```python
from build123d import *
from build123d.topology import SkipClean

# Parameters (mm, degrees)
EXTRUDE_1_DEPTH          = 12.5
HOLE_WIZARD_M14_1_D      = 12
HOLE_WIZARD_M14_1_DEPTH  = 18
SKETCH_7_W               = 66
SKETCH_7_H               = 25
EXTRUDE_2_DEPTH          = 12
CUT_EXTRUDE_1_DEPTH      = 156.608483059
CUT_EXTRUDE_1_DEPTH_BACK = 156.608483059
SKETCH_14_W              = 30
SKETCH_14_H              = 25
EXTRUDE_START            = -12.5
EXTRUDE_3_DEPTH          = 7.5
SKETCH_8_4_R             = 38.5
SKETCH_8_4_R_2           = 36.5
EXTRUDE_1_2_DEPTH        = 7.5
FILLET_1_R               = 1


with BuildPart() as part:
    # 草图1 → Extrude 1 (new, symmetric)
    with BuildSketch(Plane.XY):
        Polygon((-33, -150), (-15, -150), (-15, -100), (0, -100), (15, -100), (15, -150), (33, -150), (33, 90), (15, 90), (-15, 90), (-33, 90), align=None)
    extrude(amount=EXTRUDE_1_DEPTH, both=True)

    # M14 螺纹孔1
    with Locations(Plane(origin=(33, -131.5, 0.451602972), x_dir=(0, 0, 1), z_dir=(1, 0, 0))):
        with Locations((0, 0)):
            hole_wizard_m14_1 = Hole(HOLE_WIZARD_M14_1_D / 2, depth=HOLE_WIZARD_M14_1_DEPTH)

    # 镜向1: M14 螺纹孔1 across plane
    add(hole_wizard_m14_1.mirror(Plane(origin=(0, 0, 0), x_dir=(0, 0, 1), z_dir=(1, 0, 0))), mode=Mode.SUBTRACT)

    # 草图7 → 凸台-拉伸2 (add)
    with BuildSketch(Plane(origin=(0, 90, 0), x_dir=(1, 0, 0), z_dir=(0, 1, 0))):
        Rectangle(SKETCH_7_W, SKETCH_7_H)
    extrude(amount=EXTRUDE_2_DEPTH)

    # 草图14 → 切除-拉伸1 (cut, two sides: drawn at the far end of the back side and taken through both)
    with BuildSketch(Plane(origin=(0, 0, -12.5), x_dir=(-1, 0, 0), z_dir=(0, 0, -1)).offset(-CUT_EXTRUDE_1_DEPTH_BACK)):
        with Locations((0, 84.064537633)):
            Rectangle(SKETCH_14_W, SKETCH_14_H)
    extrude(amount=CUT_EXTRUDE_1_DEPTH + CUT_EXTRUDE_1_DEPTH_BACK, mode=Mode.SUBTRACT)

    # 草图8 → 凸台-拉伸3 (add, symmetric)
    with BuildSketch(Plane(origin=(0, 0, -12.5), x_dir=(-1, 0, 0), z_dir=(0, 0, -1)).offset(EXTRUDE_START)):
        with BuildLine():
            Line((-33, 102), (0, 102))
            Line((0, 102), (0, 125))
            ThreePointArc((0, 125), (-25.809397513, 135.690602487), (-36.5, 161.5))
            Line((-36.5, 161.5), (-36.5, 102))
            Line((-36.5, 102), (-33, 102))
        make_face()
        with BuildLine():
            Line((0, 102), (33, 102))
            Line((33, 102), (36.5, 102))
            Line((36.5, 102), (36.5, 161.5))
            ThreePointArc((36.5, 161.5), (25.809397513, 135.690602487), (0, 125))
            Line((0, 125), (0, 102))
        make_face()
    extrude(amount=EXTRUDE_3_DEPTH, both=True)

    # 草图8<4> → Extrude 1 2 (add, symmetric)
    with SkipClean():  # the faces are left unmerged after this step: merging them gives an invalid solid
        with BuildSketch(Plane(origin=(0, 0, -12.5), x_dir=(-1, 0, 0), z_dir=(0, 0, -1)).offset(EXTRUDE_START)):
            with Locations((0, 161.5)):
                Circle(SKETCH_8_4_R)
            with Locations((0, 161.5)):
                Circle(SKETCH_8_4_R_2, mode=Mode.SUBTRACT)
        extrude(amount=EXTRUDE_1_2_DEPTH, both=True)

    # 圆角1
    fillet_1_edges = [part.edges().sort_by_distance(p)[0] for p in [
        (0, 102, -7.5),
        (0, 102, 7.5),
    ]]
    fillet(fillet_1_edges, radius=FILLET_1_R)


solid = part.part
```
Could you check a few things on this model? Use its own coordinates, in mm. A direction names the side the tool comes from. Give positions to 0.01 mm unless a question says otherwise; leave off trailing zeros. Loops run counter-clockwise (first coordinate to the right, second up) from the corner with the lowest first, then second, coordinate; pieces in that order, holes last. Notation, with made-up numbers: (-21, 60) - (-16, 60) arc R23 ccw to (-16, 74) - close; hole circle Ø3 at (30.25, -15.75). An arc over 180 degrees is marked (long way). Use one line per item in the form item = value.
1. Thinking about a two-plate mould opening in X: for faces 4 (the face through (-15, -125, 0)), 5 (the face through (24, -150, 0)), 6 (the face through (-36.5, 125, 0)), which applies, released by +X, released by -X, zero draft, split by the parting line, or undercut?
Response values:
face_4 = undercut
face_5 = zero draft
face_6 = released by -X
2. On a 3-axis mill with a long thin cutter (end or side, diameter ignored), from which of +Z, -Z, +X, -X, +Y, -Y can I reach the whole of each face in a straight line? I mean faces 1 (the face through (0, -100, 0)), 2 (the face through (23.874, -125.643, 1.752)), 3 (the face through (15, 84, 0)). Say none if no direction works.
Response values:
face_1 = +Z, -Z, -Y
face_2 = +X, -X
face_3 = +Z, -Z
3. I need wall thicknesses on probe 1 along X at (y, z) = (-118, -2); probe 2 along Z at (x, y) = (-29.5, -131.5); probe 3 along Y at (x, z) = (-6.5, -9). Which ranges of each line are inside material? Lowest first, please.
Response values:
probe_1 = -33 to -15, 15 to 33
probe_2 = -12.5 to -5.55, 6.45 to 12.5
probe_3 = -100 to 71.56, 96.56 to 102
4. I want a section at C-C (x = 20). Please give me the cut outline in (y, z), and give its area (3 significant figures).
Response values:
outline = (-150, -12.5) - (102, -12.5) - (102, -8.5) arc R1 cw to (103, -7.5) - (130.97, -7.5) - (130.97, 7.5) - (103, 7.5) arc R1 cw to (102, 8.5) - (102, 12.5) - (-150, 12.5) - close; (192.03, -7.5) - (194.4, -7.5) - (194.4, 7.5) - (192.03, 7.5) - close; hole circle Ø12 at (-131.5, 0.45)
area = 6,660 mm²
5. I want a section at A-A (y = -131.5). Please give me the cut outline in (x, z), and give its area (3 significant figures).
Response values:
outline = (-33, -12.5) - (-15, -12.5) - (-15, -5.55) - (-33, -5.55) - close; (-33, 6.45) - (-15, 6.45) - (-15, 12.5) - (-33, 12.5) - close; (15, -12.5) - (33, -12.5) - (33, -5.55) - (15, -5.55) - close; (15, 6.45) - (33, 6.45) - (33, 12.5) - (15, 12.5) - close
area = 468 mm²
6. I want a section at D-D (y = 60). Please give me the cut outline in (x, z).
Response values:
outline = (-33, -12.5) - (33, -12.5) - (33, 12.5) - (-33, 12.5) - close
7. I'm going to push flat-ended pins straight in: pin 1 Ø7.5 at (x, z) = (4, 4.5) entering from +Y; pin 2 Ø4.5 at (y, z) = (121, 0) entering from -X; pin 3 Ø4 at (x, z) = (35.5, -3) entering from -Y; pin 4 Ø11 at (y, z) = (-131.5, 0.45) entering from -X. Where does each tip first touch, or does it pass through?
Response values:
pin_1 = 200
pin_2 = -36.5
pin_3 = 102
pin_4 = through
8. I want a section at B-B (x = -18). Please give me the cut outline in (y, z), and give its area (3 significant figures).
Response values:
outline = (-150, -12.5) - (102, -12.5) - (102, -8.5) arc R1 cw to (103, -7.5) - (129.75, -7.5) - (129.75, 7.5) - (103, 7.5) arc R1 cw to (102, 8.5) - (102, 12.5) - (-150, 12.5) - close; (193.25, -7.5) - (195.53, -7.5) - (195.53, 7.5) - (193.25, 7.5) - close; hole circle Ø12 at (-131.5, 0.45)
area = 6,640 mm²
